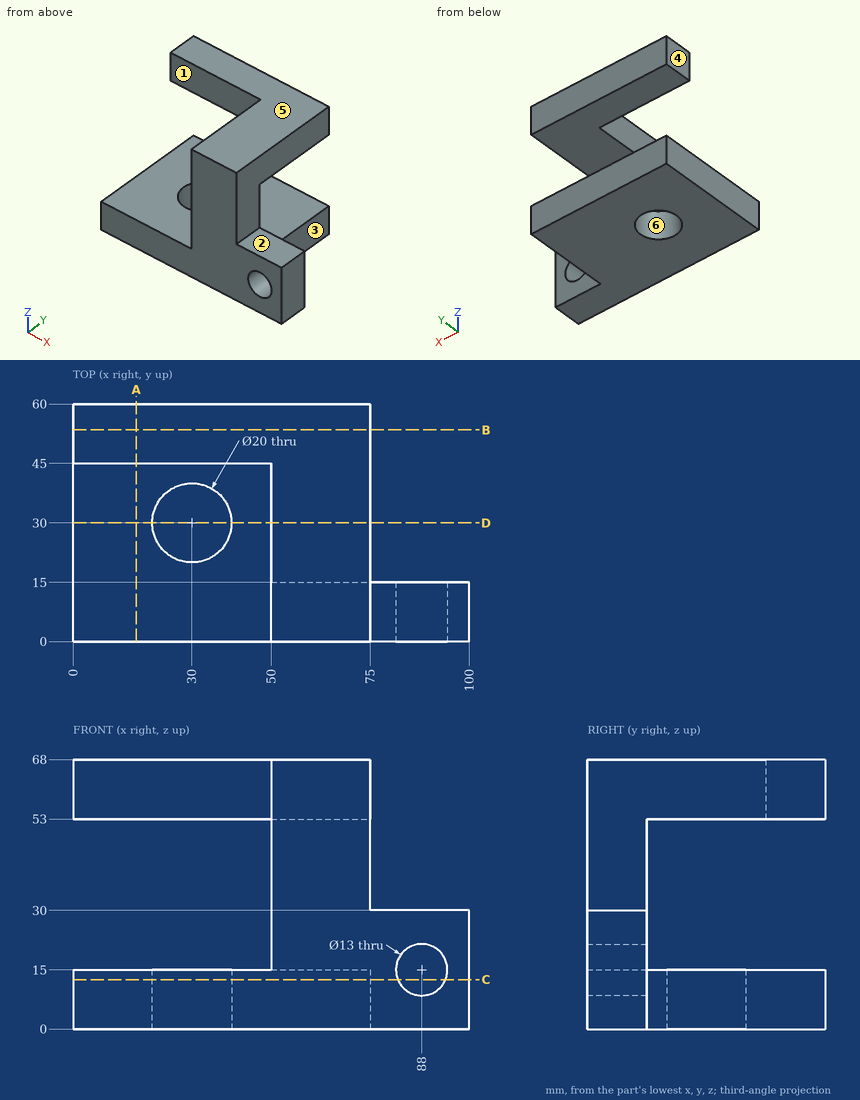
Design review of the part shown in the three views and the two pictorial views. Dimensions are in mm from the part's minimum x, y and z. A direction names the side the tool comes from. Give positions to 0.01 mm unless a question says otherwise; leave off trailing zeros. Loops run counter-clockwise (first coordinate to the right, second up) from the corner with the lowest first, then second, coordinate; pieces in that order, holes last. Notation, with made-up numbers: (75, 62) -> (96, 62) arc R13 ccw to (96, 79) -> close; hole circle Ø1 at (-29, -16). An arc over 180 degrees is marked (long way). Write each question's results on one line, items separated by ' | '.
Q1. The part is to be moulded in two halves that separate along X. For the marked faces 4, 5 and 6, say which applies: +X half, -X half, draft (parallel to the pull), parting line (faces both ways), or undercut.
Reply:
face 4: -X half | face 5: draft | face 6: undercut
Q2. Take a section at B-B, the plane y = 53.5. Write out the cut boundary in (x, z).
Reply:
outline: (0, 0) -> (75, 0) -> (75, 15) -> (0, 15) -> close; (0, 53) -> (75, 53) -> (75, 68) -> (0, 68) -> close
Q3. Machinability: for the marked faces 1, 2 and 3, which of the approach directions +Z, -Z, +X, -X, +Y, -Y give a long, thin tool a straight path to every point of the face, cutting with its end or side? Answer none if there is none.
Reply:
face 1: +Z, -X, -Y | face 2: +Z, +X, +Y, -Y | face 3: +Z, -Z, +X, +Y
Q4. Take a section at D-D, the plane y = 30. Write out the cut boundary in (x, z).
Reply:
outline: (0, 0) -> (20, 0) -> (20, 15) -> (0, 15) -> close; (40, 0) -> (75, 0) -> (75, 15) -> (40, 15) -> close; (50, 53) -> (75, 53) -> (75, 68) -> (50, 68) -> close
Q5. For pin 1 Ø11.5 at (y, z) = (38.5, 55) entering from +X; pin 2 Ø12 at (x, y) = (83, 8.5) entering from +Z; pin 3 Ø4 at (x, y) = (42, 10.5) entering from +Z, all flat-tipped, find the tip position at first contact; note any pin that passes through.
Reply:
pin 1: stops at x = 75 | pin 2: stops at z = 30 | pin 3: stops at z = 15
Q6. Wall thickness on L1, parallel to Y at x = 30, z = 11; L2, parallel to Z at x = 88, y = 3.75; L3, parallel to Z at x = 52, y = 16.5: over which ranges is each line inside the solid? List them lowest first.
Reply:
L1: y = 0 to 20, 40 to 60 | L2: z = 0 to 8.5, 21.5 to 30 | L3: z = 0 to 15, 53 to 68
Q7. Take a section at A-A, the plane x = 16. Write out the cut boundary in (y, z).
Reply:
outline: (0, 0) -> (60, 0) -> (60, 15) -> (0, 15) -> close; (45, 53) -> (60, 53) -> (60, 68) -> (45, 68) -> close
Q8. Take a section at C-C, the plane z = 12.5. Write out the cut boundary in (x, y), plus the area to 3 significant figures.
Reply:
outline: (0, 0) -> (82, 0) -> (82, 15) -> (75, 15) -> (75, 60) -> (0, 60) -> close; (94, 0) -> (100, 0) -> (100, 15) -> (94, 15) -> close; hole circle Ø20 at (30, 30) | area: 4,380 mm²
